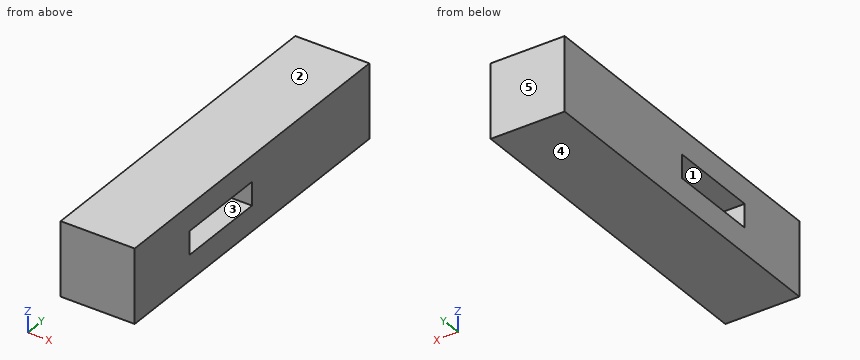
```python
from build123d import *

# Parameters (mm, degrees)
ROD_SECTION_SKETCH_38X38_W = 38
ROD_SECTION_SKETCH_38X38_H = 38
SQUARE_ROD_38X38X176_DEPTH = 176
SLOT_PROFILE_SKETCH_W      = 12
SLOT_PROFILE_SKETCH_H      = 47
THROUGH_SLOT_47X12_DEPTH   = 176


with BuildPart() as part:
    # Rod Section Sketch 38x38 → Square Rod 38x38x176 (new body)
    with BuildSketch(Plane(origin=(0, 0, 0), x_dir=(1, 0, 0), z_dir=(0, 1, 0))):
        Rectangle(ROD_SECTION_SKETCH_38X38_W, ROD_SECTION_SKETCH_38X38_H)
    extrude(amount=SQUARE_ROD_38X38X176_DEPTH)

    # Slot Profile Sketch → Through Slot 47x12 (cut)
    with BuildSketch(Plane(origin=(19, 0, 0), x_dir=(0, 0, -1), z_dir=(1, 0, 0))):
        with Locations((0, 64.5)):
            Rectangle(SLOT_PROFILE_SKETCH_W, SLOT_PROFILE_SKETCH_H)
    extrude(amount=-THROUGH_SLOT_47X12_DEPTH, mode=Mode.SUBTRACT)


solid = part.part
```
Verification items for the finished model (mm, model axes). Face numbers are marked on the shaded views. A direction names the side the tool comes from. Give positions to 0.01 mm unless a question says otherwise; leave off trailing zeros. Write each loop counter-clockwise with the first axis right and the second up, starting at its lowest first coordinate (ties: lowest second). Pieces come first, ordered by that corner, then holes. Notation, with made-up numbers: M 39.25,-6.75 L 94.25,-6.75 A25 cw 94.25,32.25 Z; hole C 33,74 d4. An arc over 180 degrees is marked long. One line per question, with ' | ' between items.
1) Thickness scan on line 1 along Y through (x, z) = (8, -3); line 2 along Z through (x, y) = (-5.5, 52.5). Record the ranges inside material, lowest first. Write a range as [from, to].
Result:
line 1: y = [0, 41], [88, 176] | line 2: z = [-19, -6], [6, 19]
2) Section check B-B on x = -5.5. Enter the section's corners in (y, z), plus the area to 3 significant figures.
Result:
outline: M 0,-19 L 176,-19 L 176,19 L 0,19 Z; hole M 41,-6 L 88,-6 L 88,6 L 41,6 Z | area: 6,120 mm2
3) Set-up check for the marked faces 1 and 2: record each of +Z, -Z, +X, -X, +Y, -Y from which the full face is reachable in a straight line by a thin tool's end or side.
Result:
face 1: +X, -X | face 2: +Z, +X, -X, +Y, -Y
4) Section check A-A on z = 4.5. Enter the section's corners in (x, y).
Result:
outline: M -19,0 L 19,0 L 19,41 L -19,41 Z; M -19,88 L 19,88 L 19,176 L -19,176 Z
5) Section check C-C on y = 79. Enter the section's corners in (x, z), plus the area to 3 significant figures.
Result:
outline: M -19,-19 L 19,-19 L 19,-6 L -19,-6 Z; M -19,6 L 19,6 L 19,19 L -19,19 Z | area: 988 mm2
6) Mould release check, pull along Y, two halves, no side actions. Record for the marked faces 3, 4 and 5: released by +Y, released by -Y, zero draft, split by the parting line, or undercut.
Result:
face 3: undercut | face 4: zero draft | face 5: released by +Y
